Verification items for the finished model (mm, model axes). A direction names the side the tool comes from. Give positions to 0.01 mm unless a question says otherwise; leave off trailing zeros. Order: outer loops, then holes, each group sorted by start corner. A loop starts at its lowest first (then second) coordinate and runs counter-clockwise, first axis right, second up. Notation, with made-up numbers: (81.25, 89.25) - (95.25, 89.25) arc R22 cw to (95.25, 114.25) - close; hole circle Ø10 at (59, 78.5). An arc over 180 degrees is marked (long way). Answer as a JSON object with one key per item and string values.
```python
from build123d import *


with BuildPart() as part:
    # Sketch1 → Revolve1 (revolve)
    with BuildSketch(Plane.XY, mode=Mode.PRIVATE) as revolve1_sk:
        Polygon((2, 7), (2, -1.5), (6, -1.5), (6, 0), (4, 0), (4, 6), (9, 6), (9, 7), align=None)
    revolve(revolve1_sk.sketch.rotate(Axis((0, 0, 0), (0, 1, 0)), 90), axis=Axis((0, 0, 0), (0, 1, 0)))


solid = part.part
```
(1) Access from +Z, -Z, +X, -X, +Y, -Y to the whole of each face (thin tool, end or side, straight path). Record for faces 4 (the cylindrical face through (3.905, 3.042, 0.867)), 5 (the cylindrical face through (-1.802, -0.74, -5.723)), 6 (the flat face through (2, 7, -2)).
Computed values:
{"face 4": "none", "face 5": "-Y", "face 6": "+Z, -Z, +X, -X, +Y"}
(2) Section check D-D (x = -2.5). Record the cut outline in (y, z), then the cut area to 3 significant figures.
Computed values:
{"outline": "(-1.5, -5.45) - (0, -5.45) - (0, -3.12) - (6, -3.12) - (6, -8.65) - (7, -8.65) - (7, 8.65) - (6, 8.65) - (6, 3.12) - (0, 3.12) - (0, 5.45) - (-1.5, 5.45) - close", "area": "71.1 mm²"}
(3) Section check C-C (y = 1). Record the cut outline in (x, z).
Computed values:
{"outline": "circle Ø8 at (0, 0); hole circle Ø4 at (0, 0)"}
(4) Release check for a two-part mould opening along X. For faces 1 (the cylindrical face through (2, 3, 0)), 2 (the flat face through (3.92, 0, 1.42)), 3 (the cylindrical face through (-6.083, 6.507, 6.633)) record: pulls with the +X half, pulls with the -X half, needs draft (parallel to the pull), parting line crosses it, or undercut.
Computed values:
{"face 1": "undercut", "face 2": "needs draft", "face 3": "parting line crosses it"}
(5) Section check A-A (z = 0). Record the cut outline in (x, y), then the cut area to 3 significant figures.
Computed values:
{"outline": "(-9, 6) - (-4, 6) - (-4, 0) - (-6, 0) - (-6, -1.5) - (-2, -1.5) - (-2, 7) - (-9, 7) - close; (2, -1.5) - (6, -1.5) - (6, 0) - (4, 0) - (4, 6) - (9, 6) - (9, 7) - (2, 7) - close", "area": "50.0 mm²"}
(6) Gauge pin test, flat ends, axial feed: pin 1 Ø5 at (y, z) = (1, 2.5) entering from -X; pin 2 Ø5 at (y, z) = (5.5, -5) entering from -X; pin 3 Ø3 at (x, y) = (2.5, 2) entering from +Z; pin 4 Ø2 at (x, y) = (6, 4.5) entering from -Z. Record the tip position at first contact, or that the pin passes through.
Computed values:
{"pin 1": "stops at x = -6", "pin 2": "stops at x = -8.63", "pin 3": "stops at z = 3.87", "pin 4": "passes through"}
(7) Section check B-B (x = 0). Record the cut outline in (y, z).
Computed values:
{"outline": "(-1.5, -6) - (0, -6) - (0, -4) - (6, -4) - (6, -9) - (7, -9) - (7, -2) - (-1.5, -2) - close; (-1.5, 2) - (7, 2) - (7, 9) - (6, 9) - (6, 4) - (0, 4) - (0, 6) - (-1.5, 6) - close"}
(8) Material ranges on line 1 along X through (y, z) = (3.5, 0); line 2 along Y through (x, z) = (5.5, 2.25); line 3 along Y through (x, z) = (-3, -7), recorded low to high. Write a range as [from, to].
Computed values:
{"line 1": "x = [-4, -2], [2, 4]", "line 2": "y = [-1.5, 0], [6, 7]", "line 3": "y = [6, 7]"}
